Part print with two shaded views. Sizes in mm from the minimum x, y, z corner. Round coordinates to 2 decimals unless told otherwise and drop trailing zeros. Loops run counter-clockwise (first coordinate to the right, second up) from the corner with the lowest first, then second, coordinate; pieces in that order, holes last. Notation, with made-up numbers: M 84.25,-29 L 143.25,-29 A13 ccw 143.25,-11 Z; hole C 8.5,19 d3. An arc over 180 degrees is marked long. Use a Markdown table: item, result. Add a question column.
Item 1: Saw through at C-C on y = 45. Write the cut outline in (x, z).
Item 2: Saw through at B-B on z = 2. Write the cut outline in (x, y).
Item 3: Two-plate mould, pull along Y, no slides. Class the marked faces 1, 2 and 3: +Y half, -Y half, draft (parallel to the pull), parting line (faces both ways), or undercut.
Item 4: Saw through at D-D on y = 10. Write the cut outline in (x, z), then the cut area to 3 significant figures.
Item 5: Wall check: L1, parallel to Y at x = 25, z = 5.5; L2, parallel to Y at x = 30, z = 1 (1 decimal); L3, parallel to Y at x = 39, z = 3.5. Give the ranges that are in metal, low to high. Write a range as from..to.
Item 6: Saw through at A-A on x = 25. Write the cut outline in (y, z).
Item 7: Pin check, flat tips, straight feed: P1, Ø3, axis at x = 25.5, z = 8.5, coming from the +Y side; P2, Ø2, axis at x = 29, z = 4.5, coming from the -Y side; P3, Ø1, axis at y = 15.5, z = 1.5, coming from the +X side; P4, Ø6, axis at y = 37, z = 5.5, coming from the +X side. Stop position of each tip, or through.
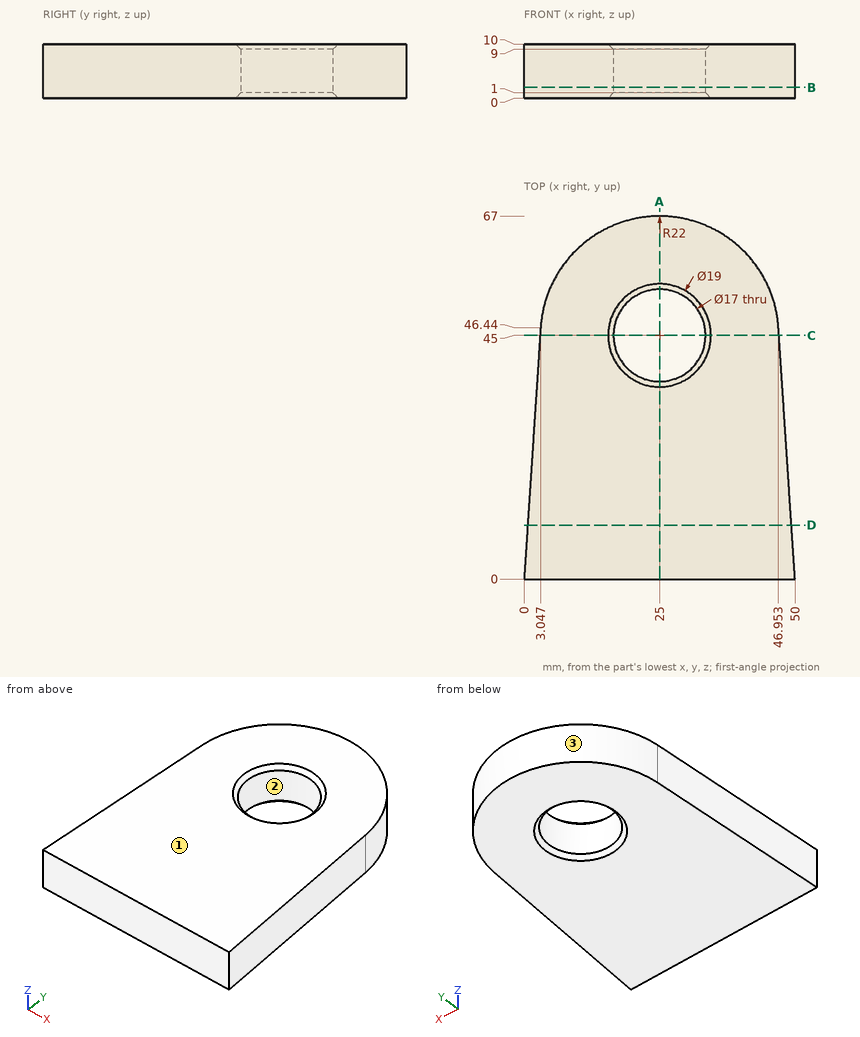
Entries:
| question | item | result |
|---|---|---|
| 1 | outline | M 2.95,0 L 15.5,0 L 16.5,1 L 16.5,9 L 15.5,10 L 2.95,10 Z; M 33.5,1 L 34.5,0 L 47.05,0 L 47.05,10 L 34.5,10 L 33.5,9 Z |
| 2 | outline | M 0,0 L 50,0 L 46.95,46.44 A22 ccw 3.05,46.44 Z; hole C 25,45 d17 |
| 3 | face 1 | draft |
| 3 | face 2 | undercut |
| 3 | face 3 | +Y half |
| 4 | outline | M 0.66,0 L 49.34,0 L 49.34,10 L 0.66,10 Z |
| 4 | area | 487 mm2 |
| 5 | L1 | 0..36.5, 53.5..67 |
| 5 | L2 | 0..38.1, 51.9..66.4 |
| 5 | L3 | 0..61.97 |
| 6 | outline | M 0,0 L 35.5,0 L 36.5,1 L 36.5,9 L 35.5,10 L 0,10 Z; M 53.5,1 L 54.5,0 L 67,0 L 67,10 L 54.5,10 L 53.5,9 Z |
| 7 | P1 | y = 67 |
| 7 | P2 | y = 0 |
| 7 | P3 | x = 49.02 |
| 7 | P4 | x = 47.77 |
